from build123d import *

# Parameters (mm, degrees)
L_BRACKET_BODY_DEPTH  = 20
UPRIGHT_HOLE_SKETCH_R = 5
UPRIGHT_HOLE_10_DEPTH = 57.789083458
BASE_HOLES_SKETCH_R   = 2.5
BASE_HOLES_2X_5_DEPTH = 57.789083458


with BuildPart() as part:
    # Bracket Profile Sketch → L-Bracket Body (new, symmetric)
    with BuildSketch(Plane.XY):
        with BuildLine():
            Line((0, 6.25), (0, 40))
            Line((0, 40), (5, 40))
            Line((5, 40), (5, 7))
            ThreePointArc((5, 7), (5.585786438, 5.585786438), (7, 5))
            Line((7, 5), (40, 5))
            Line((40, 5), (40, 0))
            Line((40, 0), (6.25, 0))
            ThreePointArc((6.25, 0), (1.830582618, 1.830582618), (0, 6.25))
        make_face()
    extrude(amount=L_BRACKET_BODY_DEPTH, both=True)

    # Upright Hole Sketch → Upright Hole Ø10 (cut, through all)
    with BuildSketch(Plane(origin=(5, 0, 0), x_dir=(0, 0, -1), z_dir=(1, 0, 0))):
        with Locations((0, 25)):
            Circle(UPRIGHT_HOLE_SKETCH_R)
    extrude(amount=-UPRIGHT_HOLE_10_DEPTH, mode=Mode.SUBTRACT)

    # Base Holes Sketch → Base Holes 2xØ5 (cut, through all)
    with BuildSketch(Plane(origin=(0, 5, 0), x_dir=(1, 0, 0), z_dir=(0, 1, 0))):
        with Locations(Location((25, 10, 0), (0, 0, 270))):
            Circle(BASE_HOLES_SKETCH_R)
        with Locations(Location((25, -10, 0), (0, 0, 270))):
            Circle(BASE_HOLES_SKETCH_R)
    extrude(amount=-BASE_HOLES_2X_5_DEPTH, mode=Mode.SUBTRACT)


solid = part.part
CAD build for the part. Positions are in the model's coordinates, mm. A direction names the side the tool comes from. Round coordinates to 2 decimals unless told otherwise and drop trailing zeros. Order: outer loops, then holes, each group sorted by start corner. A loop starts at its lowest first (then second) coordinate and runs counter-clockwise, first axis right, second up. Notation, with made-up numbers: (89.25, 9.25) -> (103.25, 9.25) arc R31 ccw to (103.25, 42.25) -> close; hole circle Ø8 at (88.5, 36.5). An arc over 180 degrees is marked (long way). Write item = value, one per line. Start each with the question number.
(1) Which spindle directions (+Z, -Z, +X, -X, +Y, -Y) get a long thin tool onto all of the face, cutting with end or side? Do faces 1 (the flat face through (23, 5, 0)), 2 (the flat face through (0, 19, 0)). Say none if no direction does.
(2) Cut at B-B, the plane y = 25. List the corners of the cut face in (x, z), then the cut area to 3 significant figures.
(3) Probe line 1 (X direction, y = 2, z = -10); line 2 (X direction, y = 10, z = -18). List the from-to ranges inside material, lowest first. Write a range as [from, to].
(4) Cut at A-A, the plane z = -10. List the corners of the cut face in (x, y).
(5) Cut at C-C, the plane x = 25. List the corners of the cut face in (y, z), then the cut area to 3 significant figures.
(6) Cut at D-D, the plane z = 14. List the corners of the cut face in (x, y), then the cut area to 3 significant figures.
(7) Pin check, flat tips, straight feed: P1, Ø4, axis at x = 25, z = 10, coming from the -Y side; P2, Ø6, axis at y = 15, z = -8.5, coming from the +X side; P3, Ø1, axis at x = 24, z = 16, coming from the +Y side. Stop position of each tip, or through.
(8) Pull direction X, two halves, no side cores. Call faces 3 (the flat face through (14, 4, -20)), 4 (the cylindrical face through (5.57, 5.6, 0.28)), 5 (the cylindrical face through (27.48, 2.54, -10.33)), 6 (the cylindrical face through (27.48, 2.54, 9.67)): released by +X, released by -X, zero draft, split by the parting line, or undercut.
Model answer:
q1.face_1 = +Z, -Z, +X, +Y
q1.face_2 = +Z, -Z, -X, +Y, -Y
q2.outline = (0, -20) -> (5, -20) -> (5, -5) -> (0, -5) -> close; (0, 5) -> (5, 5) -> (5, 20) -> (0, 20) -> close
q2.area = 150 mm2
q3.line_1 = [1.67, 22.5], [27.5, 40]
q3.line_2 = [0, 5]
q4.outline = (0, 6.25) arc R6.25 ccw to (6.25, 0) -> (22.5, 0) -> (22.5, 5) -> (7, 5) arc R2 cw to (5, 7) -> (5, 40) -> (0, 40) -> close; (27.5, 0) -> (40, 0) -> (40, 5) -> (27.5, 5) -> close
q5.outline = (0, -20) -> (5, -20) -> (5, -12.5) -> (0, -12.5) -> close; (0, -7.5) -> (5, -7.5) -> (5, 7.5) -> (0, 7.5) -> close; (0, 12.5) -> (5, 12.5) -> (5, 20) -> (0, 20) -> close
q5.area = 150 mm2
q6.outline = (0, 6.25) arc R6.25 ccw to (6.25, 0) -> (40, 0) -> (40, 5) -> (7, 5) arc R2 cw to (5, 7) -> (5, 40) -> (0, 40) -> close
q6.area = 367 mm2
q7.P1 = through
q7.P2 = 5
q7.P3 = 5
q8.face_3 = zero draft
q8.face_4 = released by +X
q8.face_5 = undercut
q8.face_6 = undercut
